Read the model definition and answer for the solid it produces. Units are mm, in the model's axes. Coordinates: 2 decimals unless noted, no trailing zeros. Order: outer loops, then holes, each group sorted by start corner. A loop starts at its lowest first (then second) coordinate and runs counter-clockwise, first axis right, second up. Notation, with made-up numbers: (-13.75, 14) -> (-1.75, 14) arc R12 cw to (-1.75, 29) -> close; hole circle Ø9 at (67.5, 73.5). An arc over 180 degrees is marked (long way). Use CSV: the item, a comma, the result in double quotes.
```python
from build123d import *


with BuildPart() as part:
    # Sketch1 → Revolve1 (revolve)
    with BuildSketch(Plane.XY, mode=Mode.PRIVATE) as revolve1_sk:
        Polygon((0, 1.97), (9.24, 1.97), (9.77, 2.5), (13.74, 2.5), (13.74, 2.1), (9.935685425, 2.1), (9.405685425, 1.57), (0, 1.57), align=None)
    revolve(revolve1_sk.sketch.rotate(Axis((0, 0, 0), (1, 0, 0)), 90), axis=Axis((0, 0, 0), (1, 0, 0)))


solid = part.part
```
Item 1: Straight lines are drawn through the part: line 1 along Y through (x, z) = (12.8, 0); line 2 along Y through (x, z) = (5.25, 0). For each, find the intervals that lie inside material, in ascending order.
Return value:
line 1,"y = -2.5 to -2.1, 2.1 to 2.5"
line 2,"y = -1.97 to -1.57, 1.57 to 1.97"
Item 2: Find section D-D, the plane x = 6. Give the vertices of the cut face in (y, z).
Return value:
outline,"circle Ø3.94 at (0, 0); hole circle Ø3.14 at (0, 0)"
Item 3: Each of these flat-tipped pins is pushed along its axis until it touches: P1, Ø2, axis at x = 12, z = -1.5, coming from the +Y side; P2, Ø3, axis at x = 8, y = 1.5, coming from the -Z side. Where does it stop, or does it pass through?
Return value:
P1,"stops at y = 2.45"
P2,"stops at z = -1.97"
Item 4: Find section C-C, the plane x = 12.5. Give the vertices of the cut face in (y, z).
Return value:
outline,"circle Ø5 at (0, 0); hole circle Ø4.2 at (0, 0)"
Item 5: The mould has two halves that part along Y. Classify faces 1 (the cylindrical face through (11.811, -0.631, 2.003)), 2 (the cylindrical face through (11.8, -0.1, -2.5)), 3 (the cylindrical face through (4.637, 1.393, 0.724)): +Y half, -Y half, draft (parallel to the pull), parting line (faces both ways), or undercut.
Return value:
face 1,"undercut"
face 2,"parting line"
face 3,"undercut"
Item 6: Find section A-A, the plane y = 0. Give the vertices of the cut face in (x, z), then the cut area to 3 significant figures.
Return value:
outline,"(0, -1.97) -> (9.24, -1.97) -> (9.77, -2.5) -> (13.74, -2.5) -> (13.74, -2.1) -> (9.94, -2.1) -> (9.41, -1.57) -> (0, -1.57) -> close; (0, 1.57) -> (9.41, 1.57) -> (9.94, 2.1) -> (13.74, 2.1) -> (13.74, 2.5) -> (9.77, 2.5) -> (9.24, 1.97) -> (0, 1.97) -> close"
area,"11.2 mm^2"
